Source: CAD feature listing. Evaluate the final solid. Frame: model axes, mm. Round coordinates to 2 decimals unless told otherwise and drop trailing zeros. Loops run counter-clockwise (first coordinate to the right, second up) from the corner with the lowest first, then second, coordinate; pieces in that order, holes last.
Item 1: Pull-direction query (X, two-part tool) for faces 1 (the cylindrical face through (-1.5, 0.07, 1.48)), 2 (the flat face through (0, -3.464, 1)), 3 (the flat face through (-2.986, 1.756, 1.479)); classes: released by +X, released by -X, zero draft, split by the parting line, or undercut.
Item 2: Section query B-B on z = 0.6. Return loops of the section in (x, y).
Item 3: Ray query, L1, parallel to Y at x = 0, z = 1.8; L2, parallel to X at y = 0.25, z = 1.15; L3, parallel to X at y = 0.5, z = 1.6. Return the intervals inside material, ascending.
Item 4: Section query D-D on x = -2.75. Return loops of the section in (y, z), then the cut area to 3 significant figures.
Item 5: Section query A-A on x = 0. Return loops of the section in (y, z), then the cut area to 3 significant figures.
Item 6: First-contact query: P1, Ø1.5, axis at x = 1, y = 0, coming from the -Z side; P2, Ø1.5, axis at y = 2, z = 1.5, coming from the +X side. Flat tips, straight axial feed; report the tip coordinate or a pass-through.
Item 7: Section query C-C on y = -2.25. Return loops of the section in (x, z).
```python
from build123d import *

# Parameters (mm, degrees)
SKETCH1_R           = 1.5
BOSS_EXTRUDE1_DEPTH = 3
CHAMFER1_SIZE       = 0.1


with BuildPart() as part:
    # Sketch1 → Boss-Extrude1 (new body)
    with BuildSketch(Plane.XY):
        Polygon((2, -3.464101615), (4, 0), (2, 3.464101615), (-2, 3.464101615), (-4, 0), (-2, -3.464101615), align=None)
        Circle(SKETCH1_R, mode=Mode.SUBTRACT)
    extrude(amount=BOSS_EXTRUDE1_DEPTH)

    # Chamfer1
    chamfer1_edges = [part.edges().sort_by_distance(p)[0] for p in [
        (-1.5, 0, 0),
        (-1.5, 0, 3),
    ]]
    chamfer(chamfer1_edges, length=CHAMFER1_SIZE)


solid = part.part
```
Data:
1. face 1: undercut
1. face 2: zero draft
1. face 3: released by -X
2. outline: (-4, 0) - (-2, -3.46) - (2, -3.46) - (4, 0) - (2, 3.46) - (-2, 3.46) - close; hole circle Ø3 at (0, 0)
3. L1: y = -3.46 to -1.5, 1.5 to 3.46
3. L2: x = -3.86 to -1.48, 1.48 to 3.86
3. L3: x = -3.71 to -1.41, 1.41 to 3.71
4. outline: (-2.17, 0) - (2.17, 0) - (2.17, 3) - (-2.17, 3) - close
4. area: 13.0 mm2
5. outline: (-3.46, 0) - (-1.6, 0) - (-1.5, 0.1) - (-1.5, 2.9) - (-1.6, 3) - (-3.46, 3) - close; (1.5, 0.1) - (1.6, 0) - (3.46, 0) - (3.46, 3) - (1.6, 3) - (1.5, 2.9) - close
5. area: 11.8 mm2
6. P1: stops at z = 0
6. P2: stops at x = 3.28
7. outline: (-2.7, 0) - (2.7, 0) - (2.7, 3) - (-2.7, 3) - close
